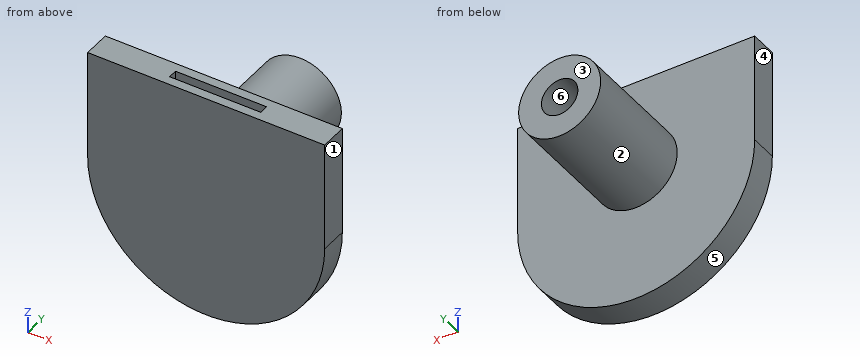
```python
from build123d import *

# Parameters (mm, degrees)
EXTRUDE_1_DEPTH     = 15
SKETCH_2_R          = 22.5
EXTRUDE_2_DEPTH     = 65
SKETCH_3_W          = 50
SKETCH_3_H          = 5
CUT_EXTRUDE_1_DEPTH = 80
SKETCH_4_R          = 10
CUT_EXTRUDE_2_DEPTH = 50


with BuildPart() as part:
    # 草图1 → 凸台-拉伸1 (new body)
    with BuildSketch(Plane(origin=(0, 0, 0), x_dir=(1, 0, 0), z_dir=(0, 1, 0))):
        with BuildLine():
            Line((0, 0), (130, 0))
            Line((130, 0), (130, 60))
            ThreePointArc((130, 60), (65, 125), (0, 60))
            Line((0, 60), (0, 0))
        make_face()
    extrude(amount=EXTRUDE_1_DEPTH)

    # 草图2 → 凸台-拉伸2 (add)
    with BuildSketch(Plane(origin=(0, 15, 0), x_dir=(1, 0, 0), z_dir=(0, 1, 0))):
        with Locations(Location((65, 50, 0), (0, 0, 270))):
            Circle(SKETCH_2_R)
    extrude(amount=EXTRUDE_2_DEPTH)

    # 草图3 → 切除-拉伸1 (cut)
    with BuildSketch(Plane.XY):
        with Locations((66.711573691, 7.5)):
            Rectangle(SKETCH_3_W, SKETCH_3_H)
    extrude(amount=-CUT_EXTRUDE_1_DEPTH, mode=Mode.SUBTRACT)

    # 草图4 → 切除-拉伸2 (cut)
    with BuildSketch(Plane(origin=(0, 80, 0), x_dir=(1, 0, 0), z_dir=(0, 1, 0))):
        with Locations(Location((65, 50, 0), (0, 0, 270))):
            Circle(SKETCH_4_R)
    extrude(amount=-CUT_EXTRUDE_2_DEPTH, mode=Mode.SUBTRACT)


solid = part.part
```
Can you work these out from the model? Positions are in its coordinate system, mm. Face numbers are marked on the shaded views. A direction names the side the tool comes from. Coordinates: 2 decimals unless noted, no trailing zeros. Write each loop counter-clockwise with the first axis right and the second up, starting at its lowest first coordinate (ties: lowest second). Pieces come first, ordered by that corner, then holes. Notation, with made-up numbers: (17.25, -31) - (52.25, -31) arc R23 cw to (52.25, 4) - close; hole circle Ø1 at (-6, 47). An arc over 180 degrees is marked (long way). Return JSON: item names as keys, results as strings.
Q1. If we section it at C-C (z = -50): Please give me the cut outline in (x, y), then the cut area to 4 significant figures.
Computed values:
{"outline": "(0, 0) - (130, 0) - (130, 15) - (87.5, 15) - (87.5, 80) - (75, 80) - (75, 30) - (55, 30) - (55, 80) - (42.5, 80) - (42.5, 15) - (0, 15) - close; hole (41.71, 5) - (91.71, 5) - (91.71, 10) - (41.71, 10) - close", "area": "3,625 mm2"}
Q2. If we section it at B-B (x = 65): Please give me the cut outline in (y, z), then the cut area to 3 significant figures.
Computed values:
{"outline": "(0, -125) - (15, -125) - (15, -72.5) - (80, -72.5) - (80, -60) - (30, -60) - (30, -40) - (80, -40) - (80, -27.5) - (15, -27.5) - (15, 0) - (10, 0) - (10, -80) - (5, -80) - (5, 0) - (0, 0) - close", "area": "3,400 mm2"}
Q3. Thinking about a two-plate mould opening in X: for the marked faces 3, 4, 5 and 6, which applies, +X half, -X half, draft (parallel to the pull), parting line (faces both ways), or undercut?
Computed values:
{"face 3": "draft", "face 4": "-X half", "face 5": "parting line", "face 6": "undercut"}
Q4. I'm going to push flat-ended pins straight in: pin 1 Ø1.5 at (y, z) = (67, -74) entering from -X; pin 2 Ø2 at (x, z) = (112, -22) entering from +Y; pin 3 Ø6 at (x, z) = (66.5, -45.5) entering from +Y; pin 4 Ø2.5 at (x, y) = (57, 7.5) entering from +Z. Where does each tip first touch, or does it pass through?
Computed values:
{"pin 1": "passes through", "pin 2": "stops at y = 15", "pin 3": "stops at y = 30", "pin 4": "stops at z = -80"}
Q5. If we section it at D-D (y = 54.5): Please give me the cut outline in (x, z), then the cut area to 3 significant figures.
Computed values:
{"outline": "circle Ø45 at (65, -50); hole circle Ø20 at (65, -50)", "area": "1,280 mm2"}
Q6. If we section it at A-A (z = -23): Please give me the cut outline in (x, y), then the cut area to 3 significant figures.
Computed values:
{"outline": "(0, 0) - (130, 0) - (130, 15) - (0, 15) - close; hole (41.71, 5) - (91.71, 5) - (91.71, 10) - (41.71, 10) - close", "area": "1,700 mm2"}
Q7. On a 3-axis mill with a long thin cutter (end or side, diameter ignored), from which of +Z, -Z, +X, -X, +Y, -Y can I reach the whole of each face in a straight line? I mean the marked faces 1 and 2. Say none if no direction works.
Computed values:
{"face 1": "+Z, -Z, +X, +Y, -Y", "face 2": "+Y"}
Q8. Please list where these lines run through material, in increasing order: L1, parallel to X at y = 52.5, z = -50; L2, parallel to Z at x = 64.5, y = 73; L3, parallel to Y at x = 67, z = -41.5. Write a range as from..to.
Computed values:
{"L1": "x = 42.5..55, 75..87.5", "L2": "z = -72.49..-59.99, -40.01..-27.51", "L3": "y = 0..5, 10..30"}
